Input: part model. Units: mm. Frame: model coordinates. Face numbers are marked on the shaded views. Coordinates: 2 decimals unless noted, no trailing zeros. Loops run counter-clockwise (first coordinate to the right, second up) from the corner with the lowest first, then second, coordinate; pieces in that order, holes last. Notation, with made-up numbers: (-20, 22.25) - (30, 22.25) arc R6 cw to (30, 30.25) - close; hole circle Ø9 at (64, 72). An arc over 180 degrees is marked (long way). Answer as CSV lines item,"result". Start each with the question number.
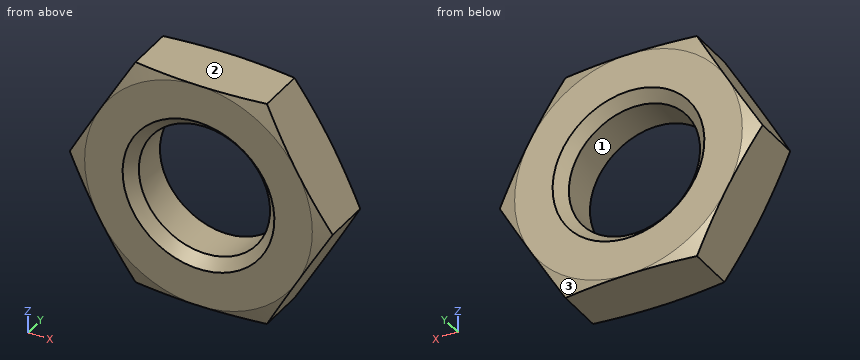
```python
from build123d import *

# Parameters (mm, degrees)
CUT_EXTRUDE_1_DEPTH      = 1.5
CUT_EXTRUDE_1_DEPTH_BACK = 1.5
SKETCH_2_R               = 12


with BuildPart() as part:
    # 草图1 → 旋转1 (revolve)
    with BuildSketch(Plane.XY, mode=Mode.PRIVATE) as revolve_1_sk:
        Polygon((3.4585, -0.9585), (4, -1.5), (6, -1.5), (9.6, -0.535382907), (9.6, 0.535382907), (6, 1.5), (4, 1.5), (3.4585, 0.9585), align=None)
    revolve(revolve_1_sk.sketch.rotate(Axis((0, -1.5, 0), (0, 1, 0)), 270), axis=Axis((0, -1.5, 0), (0, 1, 0)))

    # 草图2 → 切除-拉伸1 (cut, two sides: drawn at the far end of the back side and taken through both)
    with BuildSketch(Plane(origin=(0, 0, 0), x_dir=(1, 0, 0), z_dir=(0, 1, 0)).offset(-CUT_EXTRUDE_1_DEPTH_BACK)):
        Circle(SKETCH_2_R)
        Polygon((-6.92820323, 0), (-3.464101615, -6), (3.464101615, -6), (6.92820323, 0), (3.464101615, 6), (-3.464101615, 6), align=None, mode=Mode.SUBTRACT)
    extrude(amount=CUT_EXTRUDE_1_DEPTH + CUT_EXTRUDE_1_DEPTH_BACK, mode=Mode.SUBTRACT)


solid = part.part
```
Item 1: Material intervals for probe 1 along Z at (x, y) = (-0.75, 0.6); probe 2 along X at (y, z) = (-0.2, -0.5); probe 3 along Z at (x, y) = (-3, 0.8), sorted ascending.
Item 2: Draft query along X for the marked faces 1, 2 and 3. Return one class per face: pulls with the +X half, pulls with the -X half, needs draft (parallel to the pull), parting line crosses it, or undercut.
Item 3: Section query A-A, the plane y = -0.8. Output: boundary loops of the cut face in (x, z), and give its area (3 significant figures).
Item 4: Contact query for a flat-ended pin moving along its axis: P1, Ø6, axis at x = 0, z = -0.5, coming from the +Y side. Output: stop coordinate, or through.
Response values:
1,probe 1,"z = -6 to -3.38, 3.38 to 6"
1,probe 2,"x = -6.64 to -3.42, 3.42 to 6.64"
1,probe 3,"z = -6 to -1.72, 1.72 to 6"
2,face 1,"undercut"
2,face 2,"needs draft"
2,face 3,"pulls with the +X half"
3,outline,"(-6.93, 0) - (-3.46, -6) - (3.46, -6) - (6.93, 0) - (3.46, 6) - (-3.46, 6) - close; hole circle Ø6.92 at (0, 0)"
3,area,"87.1 mm²"
4,P1,"stops at y = 1"
